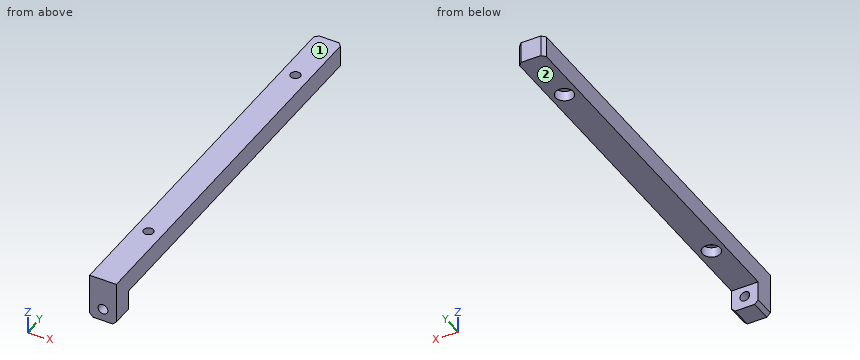
```python
from build123d import *

# Parameters (mm, degrees)
BOSS_EXTRUDE1_DEPTH                                  = 15
CBORE_FOR_M5_HEXAGON_SOCKET_HEAD_CAP_SCR_D           = 5.5
CBORE_FOR_M5_HEXAGON_SOCKET_HEAD_CAP_SCR_CBORE_D     = 10
CBORE_FOR_M5_HEXAGON_SOCKET_HEAD_CAP_SCR_CBORE_DEPTH = 5.7
M5_CLEARANCE_HOLE1_D                                 = 5.5
CHAMFER1_SIZE                                        = 2


with BuildPart() as part:
    # Sketch1 → Boss-Extrude1 (new body)
    with BuildSketch(Plane(origin=(0, 0, 0), x_dir=(0, 0, -1), z_dir=(1, 0, 0))):
        Polygon((0, 0), (25, 0), (25, 12), (12, 12), (12, 223.1), (0, 223.1), align=None)
    extrude(amount=BOSS_EXTRUDE1_DEPTH)

    # CBORE for M5 Hexagon socket head cap screws1 (through all)
    with Locations(Plane(origin=(0, 0, -12), x_dir=(-1, 0, 0), z_dir=(0, 0, -1))):
        with Locations((-7.5, 45), (-7.5, 190)):
            CounterBoreHole(CBORE_FOR_M5_HEXAGON_SOCKET_HEAD_CAP_SCR_D / 2, CBORE_FOR_M5_HEXAGON_SOCKET_HEAD_CAP_SCR_CBORE_D / 2, CBORE_FOR_M5_HEXAGON_SOCKET_HEAD_CAP_SCR_CBORE_DEPTH)

    # M5 Clearance Hole1 (through all)
    with Locations(Plane(origin=(0, 0, 0), x_dir=(-1, 0, 0), z_dir=(0, -1, 0))):
        with Locations((-7.5, 18)):
            Hole(M5_CLEARANCE_HOLE1_D / 2)

    # Chamfer1
    chamfer1_edges = [part.edges().sort_by_distance(p)[0] for p in [
        (15, 6, -25),
        (15, 223.1, -6),
        (0, 223.1, -6),
        (0, 6, -25),
    ]]
    chamfer(chamfer1_edges, length=CHAMFER1_SIZE)


solid = part.part
```
Verification items for the finished model (mm, model axes). Face numbers are marked on the shaded views. A direction names the side the tool comes from. Give positions to 0.01 mm unless a question says otherwise; leave off trailing zeros. Order: outer loops, then holes, each group sorted by start corner. A loop starts at its lowest first (then second) coordinate and runs counter-clockwise, first axis right, second up. Notation, with made-up numbers: M 59,-33.5 L 66,-33.5 A16 cw 66,-3.5 Z; hole C 84,1.5 d6. An arc over 180 degrees is marked long. Answer in a Markdown table with one row per item. Add a question column.
Item 1: Section check B-B, the plane y = 190. Enter the section's corners in (x, z).
Item 2: Scan lines: probe 1 along Y at (x, z) = (8, -10); probe 2 along Y at (x, z) = (7.5, -2.5); probe 3 along Z at (x, y) = (7.5, 8.5). Record each from-to range of solid material in increasing order. Write a range as from..to.
Item 3: Section check C-C, the plane x = 7.5. Enter the section's corners in (y, z), and give its area (3 significant figures).
Item 4: Tool access check on the marked faces 1 and 2. Record the directions out of +Z, -Z, +X, -X, +Y, -Y that give a thin tool (end or side, any length) a straight path to the whole face; none if there is none.
Item 5: Section check A-A, the plane z = -18. Enter the section's corners in (x, y), and give its area (3 significant figures).
Item 6: Section check D-D, the plane y = 108. Enter the section's corners in (x, z), and give its area (3 significant figures).
Item 7: Gauge pin test, flat ends, axial feed: pin 1 (4.5 mm diameter, centred on x = 7.5, z = -18, fed in from -Y); pin 2 (1 mm diameter, centred on x = 9.5, y = 178, fed in from -Z); pin 3 (6.5 mm diameter, centred on x = 9.5, z = -20.5, fed in from +Y); pin 4 (6 mm diameter, centred on x = 7.5, y = 190, fed in from -Z). Record the tip position at first contact, or that the pin passes through.
Filled sheet:
| question | item | result |
|---|---|---|
| 1 | outline | M 0,-12 L 2.5,-12 L 2.5,-6.3 L 4.75,-6.3 L 4.75,0 L 0,0 Z; M 10.25,-6.3 L 12.5,-6.3 L 12.5,-12 L 15,-12 L 15,0 L 10.25,0 Z |
| 2 | probe 1 | y = 0..40.03, 49.97..185.03, 194.97..223.1 |
| 2 | probe 2 | y = 0..42.25, 47.75..187.25, 192.75..223.1 |
| 2 | probe 3 | z = -25..-20.75, -15.25..0 |
| 3 | outline | M 0,-25 L 12,-25 L 12,-20.75 L 0,-20.75 Z; M 0,-15.25 L 12,-15.25 L 12,-12 L 40,-12 L 40,-6.3 L 42.25,-6.3 L 42.25,0 L 0,0 Z; M 47.75,-6.3 L 50,-6.3 L 50,-12 L 185,-12 L 185,-6.3 L 187.25,-6.3 L 187.25,0 L 47.75,0 Z; M 192.75,-6.3 L 195,-6.3 L 195,-12 L 223.1,-12 L 223.1,0 L 192.75,0 Z |
| 3 | area | 2,580 mm^2 |
| 4 | face 1 | +Z, +X, -X, +Y, -Y |
| 4 | face 2 | -Z, +X, -X, +Y |
| 5 | outline | M 0,0 L 4.75,0 L 4.75,12 L 0,12 Z; M 10.25,0 L 15,0 L 15,12 L 10.25,12 Z |
| 5 | area | 114 mm^2 |
| 6 | outline | M 0,-12 L 15,-12 L 15,0 L 0,0 Z |
| 6 | area | 180 mm^2 |
| 7 | pin 1 | passes through |
| 7 | pin 2 | stops at z = -12 |
| 7 | pin 3 | stops at y = 12 |
| 7 | pin 4 | stops at z = -6.3 |
